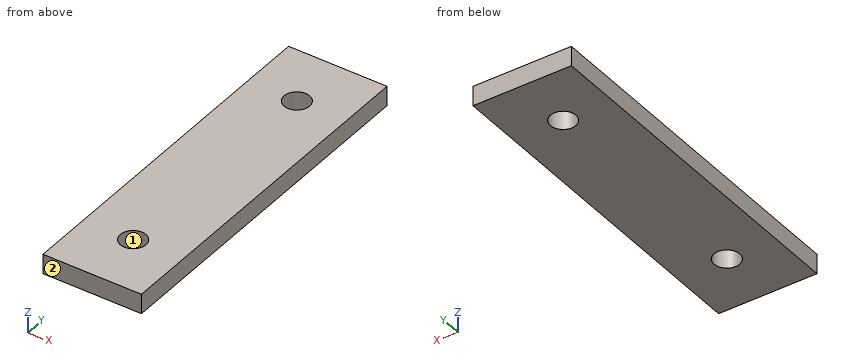
from build123d import *

# Parameters (mm, degrees)
SKETCH_1_W          = 50
SKETCH_1_H          = 180
EXTRUDE_1_DEPTH     = 10
SKETCH_2_R          = 6.5
CUT_EXTRUDE_1_DEPTH = 10


with BuildPart() as part:
    # 草图1 → 凸台-拉伸1 (new body)
    with BuildSketch(Plane.XY):
        with Locations((25, 90)):
            Rectangle(SKETCH_1_W, SKETCH_1_H)
    extrude(amount=EXTRUDE_1_DEPTH)

    # 草图2 → 切除-拉伸1 (cut)
    with BuildSketch(Plane.XY.offset(10)):
        with Locations((25, 150)):
            Circle(SKETCH_2_R)
        with Locations((25, 30)):
            Circle(SKETCH_2_R)
    extrude(amount=-CUT_EXTRUDE_1_DEPTH, mode=Mode.SUBTRACT)


solid = part.part
Can you work these out from the model? Positions are in its coordinate system, mm. Face numbers are marked on the shaded views. Give positions to 0.01 mm unless a question says otherwise; leave off trailing zeros. Loops run counter-clockwise (first coordinate to the right, second up) from the corner with the lowest first, then second, coordinate; pieces in that order, holes last. Notation, with made-up numbers: (66, -30.5) - (102, -30.5) arc R22 cw to (102, -24.5) - close; hole circle Ø11 at (1, -15). An arc over 180 degrees is marked (long way). One line per item, written item: value.
(1) I need wall thicknesses on line 1 along Y through (x, z) = (25, 4); line 2 along Y through (x, z) = (28.5, 7.25); line 3 along X through (y, z) = (150.5, 5.5). Which ranges of each line are inside material? Lowest first, please.
Verdict:
line 1: 0 to 23.5, 36.5 to 143.5, 156.5 to 180
line 2: 0 to 24.52, 35.48 to 144.52, 155.48 to 180
line 3: 0 to 18.52, 31.48 to 50
(2) If we section it at A-A, the plane y = 150: List the corners of the cut face in (x, z) for me.
Verdict:
outline: (0, 0) - (18.5, 0) - (18.5, 10) - (0, 10) - close; (31.5, 0) - (50, 0) - (50, 10) - (31.5, 10) - close
(3) If we mould it in two halves opening along X, with no side actions, what happens to the marked faces 1 and 2? For each: released by +X, released by -X, zero draft, split by the parting line, or undercut.
Verdict:
face 1: undercut
face 2: zero draft
(4) If we section it at C-C, the plane z = 5.5: List the corners of the cut face in (x, y) for me, plus the area to 3 significant figures.
Verdict:
outline: (0, 0) - (50, 0) - (50, 180) - (0, 180) - close; hole circle Ø13 at (25, 30); hole circle Ø13 at (25, 150)
area: 8,730 mm^2
(5) If we section it at B-B, the plane x = 24: List the corners of the cut face in (y, z) for me, plus the area to 3 significant figures.
Verdict:
outline: (0, 0) - (23.58, 0) - (23.58, 10) - (0, 10) - close; (36.42, 0) - (143.58, 0) - (143.58, 10) - (36.42, 10) - close; (156.42, 0) - (180, 0) - (180, 10) - (156.42, 10) - close
area: 1,540 mm^2
(6) I'm going to push a flat-ended pin straight in: pin 1 (8 mm diameter, centred on x = 25, y = 30, fed in from +Z). Where does the tip first touch, or does it pass through?
Verdict:
pin 1: through
